Here's how the part is built. I have some questions about the finished solid (model axes, mm). Face numbers are marked on the shaded views. A direction names the side the tool comes from. Round coordinates to 2 decimals unless told otherwise and drop trailing zeros. Order: outer loops, then holes, each group sorted by start corner. A loop starts at its lowest first (then second) coordinate and runs counter-clockwise, first axis right, second up. Notation, with made-up numbers: M 76.5,-25 L 117.5,-25 A17 cw 117.5,-10 Z; hole C 69,77.25 d9. An arc over 180 degrees is marked long. Use one line per item in the form item = value. Start each with the question number.
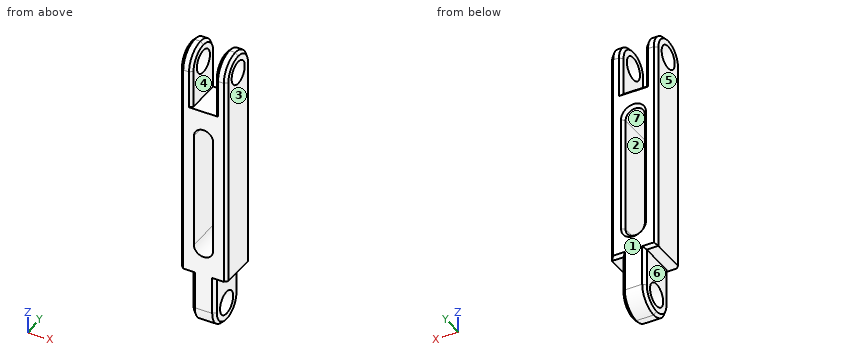
```python
from build123d import *

# Parameters (mm, degrees)
BOSS_EXTRUDE1_DEPTH = 14
SKETCH2_R           = 4
CUT_EXTRUDE1_DEPTH  = 14
SKETCH3_R           = 4
CUT_EXTRUDE2_DEPTH  = 30
CUT_EXTRUDE3_DEPTH  = 14
CHAMFER1_SIZE       = 1
SCALE1_SCALE        = 0.5


with BuildPart() as part:
    # Sketch1 → Boss-Extrude1 (new body)
    with BuildSketch(Plane(origin=(0, 0, 0), x_dir=(1, 0, 0), z_dir=(0, 1, 0))):
        Polygon((4, 40), (8, 40), (8, -40), (4, -40), (4, -20), (-4, -20), (-4, -40), (-8, -40), (-8, 40), (-4, 40), (-4, 60), (4, 60), align=None)
    extrude(amount=BOSS_EXTRUDE1_DEPTH)

    # Sketch2 → Cut-Extrude1 (cut)
    with BuildSketch(Plane(origin=(4, 0, 0), x_dir=(0, 0, -1), z_dir=(1, 0, 0))):
        with BuildLine():
            Line((60, 14), (53, 14))
            ThreePointArc((53, 14), (57.949747468, 11.949747468), (60, 7))
            Line((60, 7), (60, 14))
        make_face()
        with BuildLine():
            Line((60, 0), (60, 7))
            ThreePointArc((60, 7), (57.949747468, 2.050252532), (53, 0))
            Line((53, 0), (60, 0))
        make_face()
        with Locations((53, 7)):
            Circle(SKETCH2_R)
    extrude(amount=-CUT_EXTRUDE1_DEPTH, mode=Mode.SUBTRACT)

    # Sketch3 → Cut-Extrude2 (cut)
    with BuildSketch(Plane(origin=(8, 0, 0), x_dir=(0, 0, -1), z_dir=(1, 0, 0))):
        with BuildLine():
            ThreePointArc((-40, 7), (-37.949747468, 11.949747468), (-33, 14))
            Line((-33, 14), (-40, 14))
            Line((-40, 14), (-40, 7))
        make_face()
        with BuildLine():
            ThreePointArc((-33, 0), (-37.949747468, 2.050252532), (-40, 7))
            Line((-40, 7), (-40, 0))
            Line((-40, 0), (-33, 0))
        make_face()
        with Locations((-33, 7)):
            Circle(SKETCH3_R)
    extrude(amount=-CUT_EXTRUDE2_DEPTH, mode=Mode.SUBTRACT)

    # Sketch4 → Cut-Extrude3 (cut)
    with BuildSketch(Plane(origin=(0, 14, 0), x_dir=(1, 0, 0), z_dir=(0, 1, 0))):
        with BuildLine():
            Line((3.320010274, 30), (3.320010274, -10))
            ThreePointArc((3.320010274, -10), (0, -13.320010274), (-3.320010274, -10))
            Line((-3.320010274, -10), (-3.320010274, 30))
            ThreePointArc((-3.320010274, 30), (0, 33.320010274), (3.320010274, 30))
        make_face()
    extrude(amount=-CUT_EXTRUDE3_DEPTH, mode=Mode.SUBTRACT)

    # Chamfer1
    chamfer1_edges = [part.edges().sort_by_distance(p)[0] for p in [
        (6, 14, -40),
        (4, 0, 26.5),
        (-8, 0, -3.5),
        (4, 14, -46.5),
        (4, 0, -46.5),
        (0, 14, -33.320010274),
        (-3.320010274, 14, -10),
        (0, 14, 13.320010274),
        (3.320010274, 14, -10),
        (-6, 14, -40),
        (-8, 14, -3.5),
        (0, 14, 20),
        (-4, 14, -46.5),
        (4, 14, 26.5),
        (4, 7, -60),
        (-4, 7, -60),
        (-4, 0, -46.5),
        (4, 7, 40),
        (-4, 14, 26.5),
        (8, 14, -3.5),
        (-8, 7, 40),
        (8, 7, 40),
        (-4, 7, 40),
        (8, 0, -3.5),
        (-4, 0, 26.5),
    ]]
    chamfer(chamfer1_edges, length=CHAMFER1_SIZE)


with BuildPart() as part_1:
    # Scale1: scaled about (0, 0, 0)
    add(part.part.scale(SCALE1_SCALE))


solid = part_1.part
```
1) On a 3-axis mill with a long thin cutter (end or side, diameter ignored), from which of +Z, -Z, +X, -X, +Y, -Y can I reach the whole of each face in a straight line? I mean the marked faces 5, 6 and 7. Say none if no direction works.
2) If we mould it in two halves opening along X, with no side actions, what happens to the marked faces 1, 2, 3 and 4? For each: +X half, -X half, draft (parallel to the pull), parting line (faces both ways), or undercut.
3) If we section it at C-C on z = 10.5: Write out the boundary of the cut face in (x, y), then the cut area to 3 significant figures.
4) If I drill on line 1 (X direction, y = 3.25, z = -9.5); line 2 (X direction, y = 0.5, z = 14); line 3 (Z direction, x = -1, y = 4) (1 decimal), over which ranges is the centre line in solid material (lowest first)?
5) If we section it at B-B on x = 0.25: Give the number of separate pieces and of enclosed holes in the cut face, then the cut area to 3 significant figures.
6) Will these pins go through, and if not, where does the flat tip stop? pin 1 Ø3 at (x, y) = (2.5, 2) entering from -Z; pin 2 Ø1.5 at (x, y) = (0.5, 2.5) entering from +Z; pin 3 Ø1.2 at (x, y) = (-3, 4) entering from -Z.
7) If we section it at A-A on z = -0.5: Write out the boundary of the cut face in (x, y), then the cut area to 3 significant figures.
Completed:
q1.face_5 = +Z, -Z, -X, +Y, -Y
q1.face_6 = -Z, -X, +Y, -Y
q1.face_7 = +Y, -Y
q2.face_1 = draft
q2.face_2 = undercut
q2.face_3 = +X half
q2.face_4 = undercut
q3.outline = M -4,0.5 L -3.5,0 L -2.5,0 L -2,0.5 L -2,6.5 L -2.5,7 L -3.5,7 L -4,6.5 Z; M 2,0.5 L 2.5,0 L 3.5,0 L 4,0.5 L 4,6.5 L 3.5,7 L 2.5,7 L 2,6.5 Z
q3.area = 27.0 mm²
q4.line_1 = -4 to -1.66, 1.66 to 4
q4.line_2 = -4 to -2, 2 to 4
q4.line_3 = -30 to -28.4, -24.6 to -16.3, 6.3 to 10
q5.separate_pieces = 2
q5.enclosed_holes = 1
q5.area = 98.8 mm²
q6.pin_1 = -29.98
q6.pin_2 = 10
q6.pin_3 = -20
q7.outline = M -4,0.5 L -3.5,0 L -1.66,0 L -1.66,6.5 L -2.16,7 L -3.5,7 L -4,6.5 Z; M 1.66,0 L 3.5,0 L 4,0.5 L 4,6.5 L 3.5,7 L 2.16,7 L 1.66,6.5 Z
q7.area = 32.0 mm²
